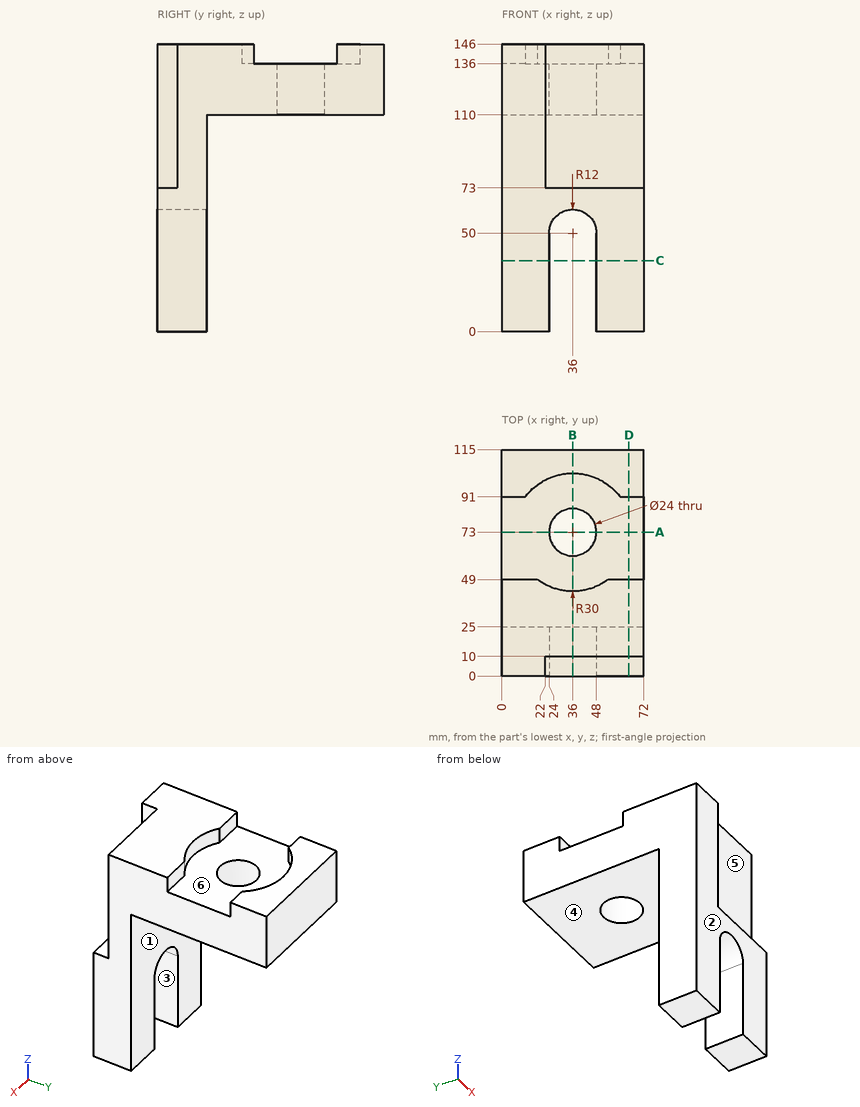
Drawing for the job (mm, zero at the part's lowest x, y, z). A direction names the side the tool comes from. Coordinates: 2 decimals unless noted, no trailing zeros. Loops run counter-clockwise (first coordinate to the right, second up) from the corner with the lowest first, then second, coordinate; pieces in that order, holes last. Notation, with made-up numbers: (-31.5, 28) - (6.5, 28) arc R21 ccw to (6.5, 44) - close; hole circle Ø6 at (-10.5, -17). An arc over 180 degrees is marked (long way). Use CSV: the item, a comma, the result in double quotes. Start each with the question number.
Q1. Two-plate mould, pull along Y, no slides. Class the marked faces 4, 5 and 6: +Y half, -Y half, draft (parallel to the pull), parting line (faces both ways), or undercut.
Q2. Cut at A-A, the plane y = 73. List the corners of the cut face in (x, z), then the cut area to 3 significant figures.
Q3. Cut at B-B, the plane x = 36. List the corners of the cut face in (y, z), then the cut area to 3 significant figures.
Q4. Probe probe 1 along Y at (x, z) = (36, 122.25); probe 2 along X at (y, z) = (9.5, 17.5); probe 3 along Y at (x, z) = (12.5, 34.5). List the from-to ranges inside material, lowest first. Write a range as from..to.
Q5. Cut at C-C, the plane z = 36. List the corners of the cut face in (x, y).
Q6. 3-axis set-ups, long thin cutter, end or side, ignore diameter. For the marked faces 1, 2 and 3: which of +Z, -Z, +X, -X, +Y, -Y reach the whole face in a straight line?
Q7. Drop flat-ended pins along their axis: P1, Ø4, axis at x = 46, y = 37.5, coming from the -Z side; P2, Ø5, axis at x = 65.5, z = 141.5, coming from the -Y side; P3, Ø2, axis at x = 53, y = 93, coming from the +Z side. Give the stop position or say it passes through.
Q8. Cut at D-D, the plane x = 64.5. List the corners of the cut face in (y, z), then the cut area to 3 significant figures.
Here are the results:
1,face 4,"draft"
1,face 5,"-Y half"
1,face 6,"undercut"
2,outline,"(0, 110) - (24, 110) - (24, 136) - (0, 136) - close; (48, 110) - (72, 110) - (72, 136) - (48, 136) - close"
2,area,"1,250 mm2"
3,outline,"(0, 62) - (25, 62) - (25, 110) - (61, 110) - (61, 136) - (43, 136) - (43, 146) - (10, 146) - (10, 73) - (0, 73) - close; (85, 110) - (115, 110) - (115, 146) - (103, 146) - (103, 136) - (85, 136) - close"
3,area,"3,390 mm2"
4,probe 1,"10..61, 85..115"
4,probe 2,"0..24, 48..72"
4,probe 3,"0..25"
5,outline,"(0, 0) - (24, 0) - (24, 25) - (0, 25) - close; (48, 0) - (72, 0) - (72, 25) - (48, 25) - close"
6,face 1,"-Z, +X, -X, +Y"
6,face 2,"+Z, -Z, +X, -X, -Y"
6,face 3,"-Z, +Y, -Y"
7,P1,"z = 110"
7,P2,"y = 10"
7,P3,"z = 136"
8,outline,"(0, 0) - (25, 0) - (25, 110) - (115, 110) - (115, 146) - (91, 146) - (91, 136) - (49, 136) - (49, 146) - (10, 146) - (10, 73) - (0, 73) - close"
8,area,"5,740 mm2"
